Could you check a few things on this model? Use its own coordinates, in mm. A direction names the side the tool comes from. Give positions to 0.01 mm unless a question says otherwise; leave off trailing zeros. Order: outer loops, then holes, each group sorted by start corner. A loop starts at its lowest first (then second) coordinate and runs counter-clockwise, first axis right, second up. Notation, with made-up numbers: M 65.5,49 L 116.5,49 A30 cw 116.5,80 Z; hole C 20.5,-24.75 d10. An arc over 180 degrees is marked long. Use a Markdown table: item, result. Add a question column.
Item 1: Suppose I cut it at B-B on y = 2.5. Count the separate pieces of the cut face and the enclosed holes in it, plus the area to 3 significant figures.
Item 2: I'm going to push flat-ended pins straight in: pin 1 Ø5 at (x, z) = (0, 60) entering from -Y; pin 2 Ø8 at (x, z) = (-6.5, 28.5) entering from +Y; pin 3 Ø10 at (y, z) = (4, 27.5) entering from -X; pin 4 Ø2.5 at (x, y) = (0, 0) entering from -Z. Where does each tip first touch, or does it pass through?
Item 3: Suppose I cut it at A-A on z = 26. Write out the boundary of the cut face in (x, y).
Item 4: If we mould it in two halves opening along X, with no side actions, what happens to faces 5 (the face through (-12.932, 5.362, 10.944)), 6 (the face through (0, -3, 0)), 7 (the face through (0.12, -2.745, 11.231))? For each: released by +X, released by -X, zero draft, split by the parting line, or undercut.
Item 5: For faces 1 (the face through (-1.5, 0.07, 61.46)), 2 (the face through (-0.9, -1.4, 9.8)), 3 (the face through (-14.985, 0.66, 23.134)), 4 (the face through (-12.932, 5.362, 59.944)), which set-ups out of +Z, -Z, +X, -X, +Y, -Y let a thin tool reach every point of the face, with its end or its side?
Item 6: If I drill on L1, parallel to Y at x = 0, z = 9.3; L2, parallel to X at y = 0, z = 2.25; L3, parallel to Z at x = -0.5, y = 8.5, over which ranges is the centre line in solid material (lowest first)? Write a range as from..to.
from build123d import *

# Parameters (mm, degrees)
SKETCH1_R                  = 15
BOSS_EXTRUDE1_DEPTH        = 71
CHAMFER1_SIZE              = 1
SKETCH6_R                  = 1.5
CUT_EXTRUDE1_DEPTH         = 17
SIZE_MM_DOWEL_HOLE_6_D     = 3
SIZE_MM_DOWEL_HOLE_6_DEPTH = 17
SIZE_MM_DOWEL_HOLE_6_TIP   = 0.901290929
SKETCH17_W                 = 2
SKETCH17_H                 = 8
SIZE_MM_DOWEL_HOLE_7_D     = 3
SIZE_MM_DOWEL_HOLE_7_DEPTH = 62
SIZE_MM_DOWEL_HOLE_7_TIP   = 0.901290929
M4_TAPPED_HOLE1_D          = 3.3
M4_TAPPED_HOLE1_DEPTH      = 5.008579979
M4_TAPPED_HOLE1_TIP        = 0.991420021


with BuildPart() as part:
    # Sketch1 → Boss-Extrude1 (new body)
    with BuildSketch(Plane.XY):
        Circle(SKETCH1_R)
    extrude(amount=BOSS_EXTRUDE1_DEPTH)

    # Chamfer1
    chamfer1_edges = [part.edges().sort_by_distance(p)[0] for p in [
        (-15, 0, 0),
        (-15, 0, 71),
    ]]
    chamfer(chamfer1_edges, length=CHAMFER1_SIZE)

    # Sketch6 → Cut-Extrude1 (cut)
    with BuildSketch(Plane(origin=(0, 15, 0), x_dir=(1, 0, 0), z_dir=(0, 1, 0))):
        with Locations(Location((0, -11, 0), (0, 0, 270))):
            Circle(SKETCH6_R)
        with Locations(Location((0, -35.5, 0), (0, 0, 270))):
            Circle(SKETCH6_R)
        with Locations(Location((0, -60, 0), (0, 0, 270))):
            Circle(SKETCH6_R)
    extrude(amount=-CUT_EXTRUDE1_DEPTH, mode=Mode.SUBTRACT)

    # Size mm dowel hole 6
    with Locations(Plane(origin=(0, 15, 0), x_dir=(1, 0, 0), z_dir=(0, 1, 0))):
        with Locations((0, -11), (0, -35.5), (0, -60)):
            Hole(SIZE_MM_DOWEL_HOLE_6_D / 2, depth=SIZE_MM_DOWEL_HOLE_6_DEPTH)
            with Locations((0, 0, -(SIZE_MM_DOWEL_HOLE_6_DEPTH + SIZE_MM_DOWEL_HOLE_6_TIP / 2))):  # 118° drill point
                Cone(0, SIZE_MM_DOWEL_HOLE_6_D / 2, SIZE_MM_DOWEL_HOLE_6_TIP, mode=Mode.SUBTRACT)

    # Sketch17 → Cut-Revolve1 (revolve, cut)
    with BuildSketch(Plane(origin=(0, 0, 0), x_dir=(1, 0, 0), z_dir=(0, 1, 0)), mode=Mode.PRIVATE) as cut_revolve1_sk:
        with Locations((15, -11)):
            Rectangle(SKETCH17_W, SKETCH17_H)
        with Locations((15, -35.5)):
            Rectangle(SKETCH17_W, SKETCH17_H)
        with Locations((15, -60)):
            Rectangle(SKETCH17_W, SKETCH17_H)
    revolve(cut_revolve1_sk.sketch.rotate(Axis((0, 0, 0), (0, 0, 1)), 180), axis=Axis((0, 0, 0), (0, 0, 1)), mode=Mode.SUBTRACT)

    # Size mm dowel hole 7
    with Locations(Plane(origin=(0, 0, 0), x_dir=(-1, 0, 0), z_dir=(0, 0, -1))):
        with Locations((0, 0)):
            Hole(SIZE_MM_DOWEL_HOLE_7_D / 2, depth=SIZE_MM_DOWEL_HOLE_7_DEPTH)
            with Locations((0, 0, -(SIZE_MM_DOWEL_HOLE_7_DEPTH + SIZE_MM_DOWEL_HOLE_7_TIP / 2))):  # 118° drill point
                Cone(0, SIZE_MM_DOWEL_HOLE_7_D / 2, SIZE_MM_DOWEL_HOLE_7_TIP, mode=Mode.SUBTRACT)

    # M4 Tapped Hole1
    with Locations(Plane(origin=(0, 0, 0), x_dir=(-1, 0, 0), z_dir=(0, 0, -1))):
        with Locations((0, 0)):
            Hole(M4_TAPPED_HOLE1_D / 2, depth=M4_TAPPED_HOLE1_DEPTH)
            with Locations((0, 0, -(M4_TAPPED_HOLE1_DEPTH + M4_TAPPED_HOLE1_TIP / 2))):  # 118° drill point
                Cone(0, M4_TAPPED_HOLE1_D / 2, M4_TAPPED_HOLE1_TIP, mode=Mode.SUBTRACT)


solid = part.part
Findings below:
| question | item | result |
|---|---|---|
| 1 | separate pieces | 1 |
| 1 | enclosed holes | 3 |
| 1 | area | 2,030 mm^2 |
| 2 | pin 1 | stops at y = -14 |
| 2 | pin 2 | stops at y = 14.79 |
| 2 | pin 3 | stops at x = -15 |
| 2 | pin 4 | stops at z = 62.15 |
| 3 | outline | C 0,0 d30; hole C 0,0 d3 |
| 4 | face 5 | split by the parting line |
| 4 | face 6 | zero draft |
| 4 | face 7 | undercut |
| 5 | face 1 | -Z |
| 5 | face 2 | +Y |
| 5 | face 3 | +Z, -Z |
| 5 | face 4 | none |
| 6 | L1 | y = -14..-1.5, 1.5..14 |
| 6 | L2 | x = -15..-1.65, 1.65..15 |
| 6 | L3 | z = 0..9.59, 12.41..34.09, 36.91..58.59, 61.41..71 |
